from build123d import *

# Parameters (mm, degrees)
SKETCH1_W            = 230
SKETCH1_H            = 160
BOSS_EXTRUDE1_DEPTH  = 20
SKETCH4_R            = 50
CUT_EXTRUDE3_DEPTH   = 109
SKETCH5_R            = 10.25
CUT_EXTRUDE4_DEPTH   = 6
M8_CLEARANCE_HOLE1_D = 9
CHAMFER2_SIZE        = 1
CUT_EXTRUDE6_DEPTH   = 214
FILLET1_R            = 15
CHAMFER3_SIZE        = 1
CHAMFER4_SIZE        = 1
M5_TAPPED_HOLE1_D    = 4.2


with BuildPart() as part:
    # Sketch1 → Boss-Extrude1 (new body)
    with BuildSketch(Plane.XY):
        Rectangle(SKETCH1_W, SKETCH1_H)
    extrude(amount=BOSS_EXTRUDE1_DEPTH)

    # Sketch4 → Cut-Extrude3 (cut)
    with BuildSketch(Plane.XY.offset(20)):
        Circle(SKETCH4_R)
    extrude(amount=-CUT_EXTRUDE3_DEPTH, mode=Mode.SUBTRACT)

    # Sketch5 → Cut-Extrude4 (cut)
    with BuildSketch(Plane.XY):
        with Locations((-95, 0)):
            Circle(SKETCH5_R)
        with Locations((95, 0)):
            Circle(SKETCH5_R)
    extrude(amount=CUT_EXTRUDE4_DEPTH, mode=Mode.SUBTRACT)

    # M8 Clearance Hole1 (through all)
    with Locations(Plane.XY.offset(20)):
        with Locations((-95, 0), (95, 0)):
            Hole(M8_CLEARANCE_HOLE1_D / 2)

    # Chamfer2
    chamfer2_edges = [part.edges().sort_by_distance(p)[0] for p in [
        (-50, 0, 0),
        (-50, 0, 20),
    ]]
    chamfer(chamfer2_edges, length=CHAMFER2_SIZE)

    # Sketch10 → Cut-Extrude6 (cut)
    with BuildSketch(Plane.XY.offset(20)):
        Polygon((-115, 80), (-35, 80), (-115, 15), align=None)
        Polygon((35, 80), (115, 80), (115, 15), align=None)
        Polygon((-115, -15), (-35, -80), (-115, -80), align=None)
        Polygon((35, -80), (115, -80), (115, -15), align=None)
    extrude(amount=-CUT_EXTRUDE6_DEPTH, mode=Mode.SUBTRACT)

    # Fillet1
    fillet1_edges = [part.edges().sort_by_distance(p)[0] for p in [
        (115, 15, 10),
        (35, 80, 10),
        (-115, -15, 10),
        (-35, -80, 10),
        (35, -80, 10),
        (115, -15, 10),
        (-115, 15, 10),
        (-35, 80, 10),
    ]]
    fillet(fillet1_edges, radius=FILLET1_R)

    # Chamfer3
    chamfer3_edges = [part.edges().sort_by_distance(p)[0] for p in [
        (-74.296084687, 48.071931192, 0),
        (-74.296084687, 48.071931192, 20),
        (115, 0, 20),
        (74.296084687, 48.071931192, 20),
        (0, 80, 20),
        (-115, 0, 20),
        (-74.296084687, -48.071931192, 20),
        (0, -80, 20),
        (74.296084687, -48.071931192, 20),
        (-113.544064025, -14.307017415, 20),
        (-34.693073216, -79.13551644, 20),
        (34.693073216, -79.13551644, 20),
        (113.544064025, -14.307017415, 20),
        (113.544064025, 14.307017415, 20),
        (34.693073216, 79.13551644, 20),
        (-34.693073216, 79.13551644, 20),
        (-113.544064025, 14.307017415, 20),
        (-115, 0, 0),
        (74.296084687, 48.071931192, 0),
        (115, 0, 0),
        (74.296084687, -48.071931192, 0),
        (0, -80, 0),
        (-74.296084687, -48.071931192, 0),
        (0, 80, 0),
        (-113.544064025, -14.307017415, 0),
        (-34.693073216, -79.13551644, 0),
        (34.693073216, -79.13551644, 0),
        (113.544064025, -14.307017415, 0),
        (113.544064025, 14.307017415, 0),
        (34.693073216, 79.13551644, 0),
        (-34.693073216, 79.13551644, 0),
        (-113.544064025, 14.307017415, 0),
    ]]
    chamfer(chamfer3_edges, length=CHAMFER3_SIZE)

    # Chamfer4
    chamfer4_edges = [part.edges().sort_by_distance(p)[0] for p in [
        (-105.25, 0, 0),
        (84.75, 0, 0),
    ]]
    chamfer(chamfer4_edges, length=CHAMFER4_SIZE)

    # M5 Tapped Hole1 (through all)
    with Locations(Plane.XY.offset(20)):
        with Locations((-30, 51.961524227), (-60, 0), (-30, -51.961524227), (30, -51.961524227), (60, 0), (30, 51.961524227)):
            Hole(M5_TAPPED_HOLE1_D / 2)


solid = part.part
CAD build for the part. Positions are in the model's coordinates, mm. A direction names the side the tool comes from. Coordinates: 2 decimals unless noted, no trailing zeros. Order: outer loops, then holes, each group sorted by start corner. A loop starts at its lowest first (then second) coordinate and runs counter-clockwise, first axis right, second up.
Item 1: 3-axis set-ups, long thin cutter, end or side, ignore diameter. For faces 4 (the face through (97.1, -4.4, 6)), 5 (the face through (-112.85, 14.07, 19.73)): which of +Z, -Z, +X, -X, +Y, -Y reach the whole face in a straight line?
Check sheet entries:
face 4: -Z
face 5: +Z, -X, +Y
Item 2: Band-saw the part on C-C on x = -53.5. List the corners of the cut face in (y, z), plus the area to 3 significant figures.
Check sheet entries:
outline: (-64.97, 1) - (-63.68, 0) - (63.68, 0) - (64.97, 1) - (64.97, 19) - (63.68, 20) - (-63.68, 20) - (-64.97, 19) - close
area: 2,600 mm2
Item 3: Band-saw the part on B-B on z = 10. Give the number of separate pieces and of enclosed holes in the cut face, plus the area to 3 significant figures.
Check sheet entries:
separate pieces: 1
enclosed holes: 9
area: 18,300 mm2
Item 4: Band-saw the part on A-A on x = -95. List the corners of the cut face in (y, z).
Check sheet entries:
outline: (-31.25, 1) - (-29.96, 0) - (-11.25, 0) - (-10.25, 1) - (-10.25, 6) - (-4.5, 6) - (-4.5, 20) - (-29.96, 20) - (-31.25, 19) - close; (4.5, 6) - (10.25, 6) - (10.25, 1) - (11.25, 0) - (29.96, 0) - (31.25, 1) - (31.25, 19) - (29.96, 20) - (4.5, 20) - close
Item 5: Two-plate mould, pull along X, no slides. Class faces 1 (the face through (47.69, 15.02, 10.13)), 2 (the face through (74.79, 47.67, 10.13)), 3 (the face through (-74.79, -47.67, 10.13)): +X half, -X half, draft (parallel to the pull), parting line (faces both ways), or undercut.
Check sheet entries:
face 1: undercut
face 2: +X half
face 3: -X half
Item 6: Drill centre lines: L1, parallel to X at y = 7, z = 5.25; L2, parallel to Y at x = 30, z = 7.75; L3, parallel to X at y = 38, z = 7.5. Where is each one in solid material? Low to high.
Check sheet entries:
L1: x = -115 to -102.49, -87.51 to -49.51, 49.51 to 87.51, 102.49 to 115
L2: y = -80 to -54.06, -49.86 to -40, 40 to 49.86, 54.06 to 80
L3: x = -86.69 to -32.5, 32.5 to 86.69
Item 7: Pin check, flat tips, straight feed: pin 1 Ø11.5 at (x, y) = (-95, 0) entering from -Z; pin 2 Ø4 at (x, y) = (60, 0) entering from -Z; pin 3 Ø1 at (x, z) = (47.5, 5) entering from +Y; pin 4 Ø5.5 at (x, y) = (-60, 0) entering from -Z. Stop position of each tip, or through.
Check sheet entries:
pin 1: stops at z = 6
pin 2: passes through
pin 3: stops at y = 70.25
pin 4: stops at z = 0
